Source: CAD feature listing. Evaluate the final solid. Frame: model axes, mm. Round coordinates to 2 decimals unless told otherwise and drop trailing zeros. Loops run counter-clockwise (first coordinate to the right, second up) from the corner with the lowest first, then second, coordinate; pieces in that order, holes last. Notation, with made-up numbers: M 36.5,32.25 L 81.5,32.25 A23 cw 81.5,67.25 Z; hole C 42.5,2 d5. An arc over 180 degrees is marked long. Answer as a JSON object with one key per item and string values.
from build123d import *

# Parameters (mm, degrees)
EXTRUDE_1_DEPTH = 2


with BuildPart() as part:
    # 草图1 → 凸台-拉伸1 (new body)
    with BuildSketch(Plane.XY):
        Polygon((0, 0), (30.5, 0), (30.5, -17), (10, -48), (0, -48), align=None)
    extrude(amount=EXTRUDE_1_DEPTH)


solid = part.part
Item 1: Section C-C on y = -28. Return the cut outline in (x, z), then the cut area to 3 significant figures.
Answer sheet:
{"outline": "M 0,0 L 23.23,0 L 23.23,2 L 0,2 Z", "area": "46.5 mm²"}
Item 2: Contact query for a flat-ended pin moving along its axis: pin 1 Ø1 at (y, z) = (-19, 1) entering from +X. Output: stop coordinate, or through.
Answer sheet:
{"pin 1": "stops at x = 29.51"}
Item 3: Line query: probe 1 along X at (y, z) = (-37.5, 0.8); probe 2 along Y at (x, z) = (12.5, 1.5); probe 3 along Y at (x, z) = (17.5, 1.4). Output: solid intervals per line, ascending. Write a range as from..to.
Answer sheet:
{"probe 1": "x = 0..16.94", "probe 2": "y = -44.22..0", "probe 3": "y = -36.66..0"}
Item 4: Section A-A on z = 0.55. Return the cut outline in (x, y).
Answer sheet:
{"outline": "M 0,-48 L 10,-48 L 30.5,-17 L 30.5,0 L 0,0 Z"}
Item 5: Section B-B on x = 19. Return the cut outline in (y, z), then the cut area to 3 significant figures.
Answer sheet:
{"outline": "M -34.39,0 L 0,0 L 0,2 L -34.39,2 Z", "area": "68.8 mm²"}
